Input: dimensioned drawing with shaded views. Units: mm. Origin: part minimum x, y, z. A direction names the side the tool comes from. Round coordinates to 2 decimals unless told otherwise and drop trailing zeros. Loops run counter-clockwise (first coordinate to the right, second up) from the corner with the lowest first, then second, coordinate; pieces in that order, holes last. Notation, with made-up numbers: (10.5, -16) - (59.5, -16) arc R25 cw to (59.5, 3) - close; hole circle Ø6 at (-10.75, 78.25). An arc over 180 degrees is marked (long way). Use CSV: the item, a comma, the result in double quotes. Start each with the question number.
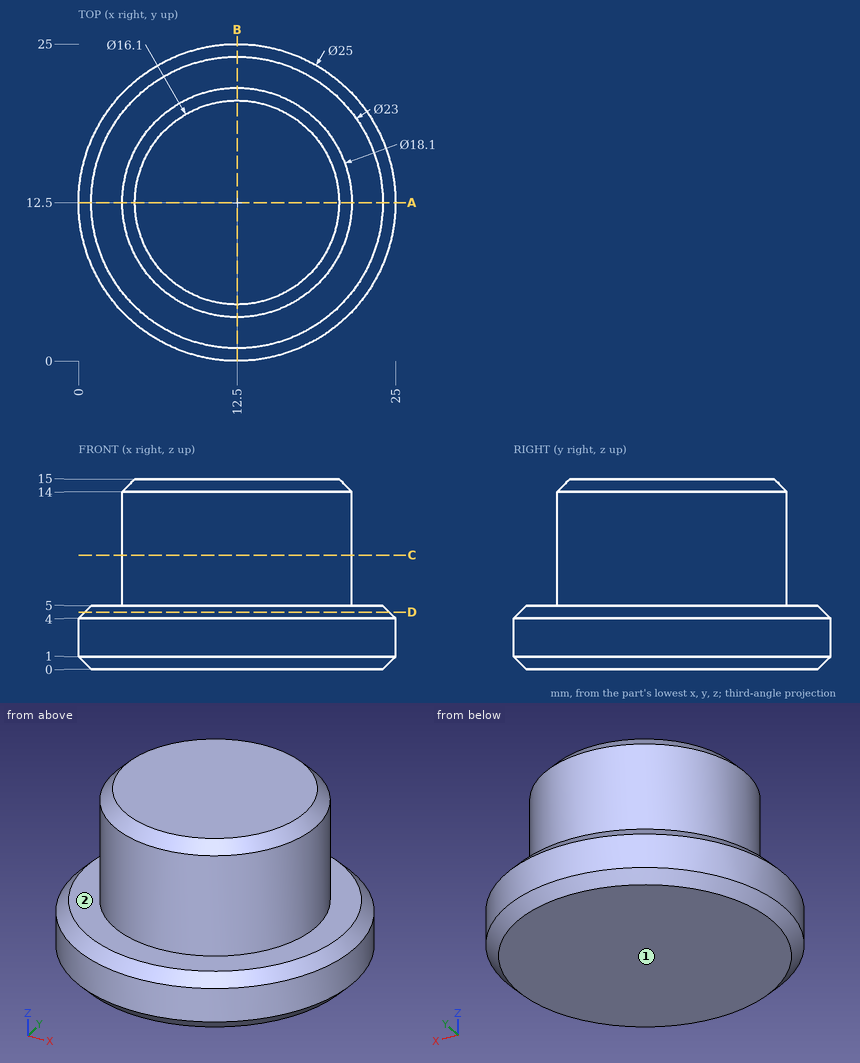
1. Line query: line 1 along X through (y, z) = (12.75, 13.75); line 2 along Z through (x, y) = (10, 3); line 3 along X through (y, z) = (4.25, 4.25). Output: solid intervals per line, ascending.
2. Contact query for flat-ended pins moving along their axis: P1, Ø1.5, axis at y = 13.5, z = 5.5, coming from the -X side; P2, Ø1, axis at x = 3.5, y = 10, coming from the +Z side; P3, Ø1, axis at x = 17, z = 12, coming from the -Y side. Output: stop coordinate, or through.
3. Section query A-A on y = 12.5. Return the cut outline in (x, z), and give its area (3 significant figures).
4. Section query D-D on z = 4.5. Return the cut outline in (x, y).
5. Reachability of the marked faces 1 and 2 from +Z, -Z, +X, -X, +Y, -Y: full face, straight path, thin tool, end or side. Return the list, or none.
6. Section query C-C on z = 9. Return the cut outline in (x, y).
Values:
1,line 1,"x = 3.45 to 21.55"
1,line 2,"z = 0 to 5"
1,line 3,"x = 3.44 to 21.56"
2,P1,"stops at x = 0.79"
2,P2,"stops at z = 14.21"
2,P3,"stops at y = 4.38"
3,outline,"(0, 1) - (1, 0) - (24, 0) - (25, 1) - (25, 4) - (24, 5) - (21.55, 5) - (21.55, 14) - (20.55, 15) - (4.45, 15) - (3.45, 14) - (3.45, 5) - (1, 5) - (0, 4) - close"
3,area,"303 mm^2"
4,outline,"circle Ø24 at (12.5, 12.5)"
5,face 1,"-Z, +X, -X, +Y, -Y"
5,face 2,"+Z"
6,outline,"circle Ø18.1 at (12.5, 12.5)"
